Input: part model. Units: mm. Frame: model coordinates. A direction names the side the tool comes from. Give positions to 0.01 mm unless a question says otherwise; leave off trailing zeros. Write each loop counter-clockwise with the first axis right and the second up, starting at its lowest first coordinate (ties: lowest second). Pieces come first, ordered by that corner, then holes. Notation, with made-up numbers: (45, 63.5) -> (73, 63.5) arc R10 ccw to (73, 73.5) -> close; hole circle Ø2 at (6, 40.25). An arc over 180 degrees is marked (long way). Answer as a JSON object with one key per item and string values. Group by question number.
from build123d import *

# Parameters (mm, degrees)
SKETCH1_R           = 50
BOSS_EXTRUDE1_DEPTH = 20
SKETCH2_R           = 52
BOSS_EXTRUDE2_DEPTH = 8
BOSS_EXTRUDE3_START = 8
SKETCH3_R           = 52
BOSS_EXTRUDE3_DEPTH = 8
SKETCH4_R           = 25
CUT_EXTRUDE1_DEPTH  = 82.877957962


with BuildPart() as part:
    # Sketch1 → Boss-Extrude1 (new body)
    with BuildSketch(Plane(origin=(0, 0, 0), x_dir=(1, 0, 0), z_dir=(0, 1, 0))):
        with Locations(Location((0, 0, 0), (0, 0, 270))):
            Circle(SKETCH1_R)
    extrude(amount=BOSS_EXTRUDE1_DEPTH)

    # Sketch2 → Boss-Extrude2 (add)
    with BuildSketch(Plane(origin=(0, 20, 0), x_dir=(1, 0, 0), z_dir=(0, 1, 0))):
        with Locations(Location((0, 0, 0), (0, 0, 270))):
            Circle(SKETCH2_R)
    extrude(amount=BOSS_EXTRUDE2_DEPTH)

    # Sketch3 → Boss-Extrude3 (add)
    with BuildSketch(Plane.XZ.offset(BOSS_EXTRUDE3_START)):
        with Locations(Location((0, 0, 0), (0, 0, 90))):
            Circle(SKETCH3_R)
    extrude(amount=-BOSS_EXTRUDE3_DEPTH)

    # Sketch4 → Cut-Extrude1 (cut, through all)
    with BuildSketch(Plane.XZ.offset(8)):
        with Locations(Location((0, 0, 0), (0, 0, 270))):
            Circle(SKETCH4_R)
    extrude(amount=-CUT_EXTRUDE1_DEPTH, mode=Mode.SUBTRACT)


solid = part.part
1. Mould query, pull axis X, two halves, no side actions, for faces 1 (the face through (7.509, 9.748, -23.846)), 2 (the face through (-12.3, -8, 22.4)), 3 (the face through (-31.641, 23.944, -41.265)). Classes: pulls with the +X half, pulls with the -X half, needs draft (parallel to the pull), parting line crosses it, or undercut.
2. Section C-C (y = 14.5). Return the cut outline in (x, z).
3. Reachability of faces 4 (the face through (12.3, 28, 22.4)), 5 (the face through (43, 20, -27)) from +Z, -Z, +X, -X, +Y, -Y: full face, straight path, thin tool, end or side. Return the list, or none.
4. Contact query for flat-ended pins moving along their axis: pin 1 Ø10 at (x, y) = (17.5, 7.5) entering from +Z; pin 2 Ø8 at (x, y) = (36, 18) entering from -Z; pin 3 Ø5 at (y, z) = (10.5, -30) entering from -X. Output: stop coordinate, or through.
5. Line query: line 1 (X direction, y = 19, z = 0); line 2 (Z direction, x = -2.5, y = 23); line 3 (Z direction, x = -12, y = 15.5). Output: solid intervals per line, ascending.
6. Section A-A (z = 0). Return the cut outline in (x, y), plus the area to 3 significant figures.
7. Section B-B (x = 0). Return the cut outline in (y, z).
8. Section D-D (z = 39). Return the cut outline in (x, y).
Working result:
{
 "1": {"face 1": "undercut", "face 2": "needs draft", "face 3": "parting line crosses it"},
 "2": {"outline": "circle Ø100 at (0, 0); hole circle Ø50 at (0, 0)"},
 "3": {"face 4": "+Z, -Z, +X, -X, +Y", "face 5": "none"},
 "4": {"pin 1": "stops at z = 48.41", "pin 2": "stops at z = -40.56", "pin 3": "stops at x = -41.76"},
 "5": {"line 1": "x = -50 to -25, 25 to 50", "line 2": "z = -51.94 to -24.87, 24.87 to 51.94", "line 3": "z = -48.54 to -21.93, 21.93 to 48.54"},
 "6": {"outline": "(-52, -8) -> (-25, -8) -> (-25, 28) -> (-52, 28) -> (-52, 20) -> (-50, 20) -> (-50, 0) -> (-52, 0) -> close; (25, -8) -> (52, -8) -> (52, 0) -> (50, 0) -> (50, 20) -> (52, 20) -> (52, 28) -> (25, 28) -> close", "area": "1,860 mm^2"},
 "7": {"outline": "(-8, -52) -> (0, -52) -> (0, -50) -> (20, -50) -> (20, -52) -> (28, -52) -> (28, -25) -> (-8, -25) -> close; (-8, 25) -> (28, 25) -> (28, 52) -> (20, 52) -> (20, 50) -> (0, 50) -> (0, 52) -> (-8, 52) -> close"},
 "8": {"outline": "(-34.39, -8) -> (34.39, -8) -> (34.39, 0) -> (31.29, 0) -> (31.29, 20) -> (34.39, 20) -> (34.39, 28) -> (-34.39, 28) -> (-34.39, 20) -> (-31.29, 20) -> (-31.29, 0) -> (-34.39, 0) -> close"}
}
